from build123d import *

# Parameters (mm, degrees)
SKETCH_1_W          = 200
SKETCH_1_H          = 150
EXTRUDE_1_DEPTH     = 10
HOLE_WIZARD_M10_1_D = 8.5


with BuildPart() as part:
    # 草图1 → 凸台-拉伸1 (new body)
    with BuildSketch(Plane(origin=(0, 0, 0), x_dir=(1, 0, 0), z_dir=(0, 1, 0))):
        Rectangle(SKETCH_1_W, SKETCH_1_H)
    extrude(amount=EXTRUDE_1_DEPTH)

    # M10 螺纹孔1 (through all)
    with Locations(Plane(origin=(0, 0, 0), x_dir=(-1, 0, 0), z_dir=(0, -1, 0))):
        with Locations((90, -65), (90, 65), (-90, 65), (-90, -65)):
            Hole(HOLE_WIZARD_M10_1_D / 2)


solid = part.part
CAD build for the part. Positions are in the model's coordinates, mm. Round coordinates to 2 decimals unless told otherwise and drop trailing zeros. Write each loop counter-clockwise with the first axis right and the second up, starting at its lowest first coordinate (ties: lowest second). Pieces come first, ordered by that corner, then holes. Notation, with made-up numbers: (55, 57) -> (59, 57) arc R21 ccw to (59, 93) -> close; hole circle Ø9 at (21, 45). An arc over 180 degrees is marked (long way). Answer as a JSON object with one key per item and string values.
(1) Two-plate mould, pull along X, no slides. Class faces 1 (the face through (86.63, 5.07, -62.41)), 2 (the face through (-1, 10, -1)), 3 (the face through (-93.37, 5.07, 67.59)), 4 (the face through (-100, 5, 1)): +X half, -X half, draft (parallel to the pull), parting line (faces both ways), or undercut.
Reported:
{"face 1": "undercut", "face 2": "draft", "face 3": "undercut", "face 4": "-X half"}
(2) Band-saw the part on B-B, the plane z = -65. List the corners of the cut face in (x, y), then the cut area to 3 significant figures.
Reported:
{"outline": "(-100, 0) -> (-94.25, 0) -> (-94.25, 10) -> (-100, 10) -> close; (-85.75, 0) -> (85.75, 0) -> (85.75, 10) -> (-85.75, 10) -> close; (94.25, 0) -> (100, 0) -> (100, 10) -> (94.25, 10) -> close", "area": "1,830 mm^2"}
(3) Probe probe 1 along X at (y, z) = (5.5, 65); probe 2 along Z at (x, y) = (-90, 7.5). List the from-to ranges inside material, lowest first. Write a range as [from, to].
Reported:
{"probe 1": "x = [-100, -94.25], [-85.75, 85.75], [94.25, 100]", "probe 2": "z = [-75, -69.25], [-60.75, 60.75], [69.25, 75]"}
(4) Band-saw the part on A-A, the plane x = 90. List the corners of the cut face in (y, z), then the cut area to 3 significant figures.
Reported:
{"outline": "(0, -75) -> (10, -75) -> (10, -69.25) -> (0, -69.25) -> close; (0, -60.75) -> (10, -60.75) -> (10, 60.75) -> (0, 60.75) -> close; (0, 69.25) -> (10, 69.25) -> (10, 75) -> (0, 75) -> close", "area": "1,330 mm^2"}
